Input: part model. Units: mm. Frame: model coordinates. Coordinates: 2 decimals unless noted, no trailing zeros. Write each loop counter-clockwise with the first axis right and the second up, starting at its lowest first coordinate (ties: lowest second). Pieces come first, ordered by that corner, then holes.
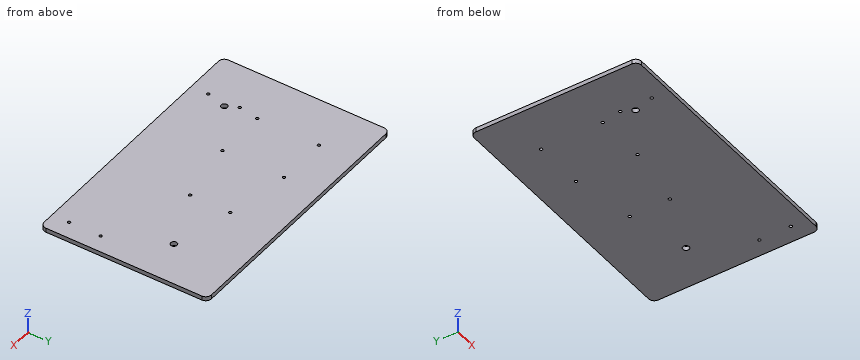
from build123d import *

# Parameters (mm, degrees)
SKETCH_1_R           = 5
SKETCH_1_R_2         = 11
BOSS_EXTRUDE_1_DEPTH = 15


with BuildPart() as part:
    # Sketch 1 → Boss-Extrude 1 (new body)
    with BuildSketch(Plane.XY):
        with BuildLine():
            Line((-465, -273), (-465, 273))
            ThreePointArc((-465, 273), (-459.142135624, 287.142135624), (-445, 293))
            Line((-445, 293), (445, 293))
            ThreePointArc((445, 293), (459.142135624, 287.142135624), (465, 273))
            Line((465, 273), (465, -273))
            ThreePointArc((465, -273), (459.142135624, -287.142135624), (445, -293))
            Line((445, -293), (-445, -293))
            ThreePointArc((-445, -293), (-459.142135624, -287.142135624), (-465, -273))
        make_face()
        with Locations((-115, 163)):
            Circle(SKETCH_1_R, mode=Mode.SUBTRACT)
        with Locations((-293, 163)):
            Circle(SKETCH_1_R, mode=Mode.SUBTRACT)
        with Locations(Location((-293, -53, 0), (0, 0, 180))):
            Circle(SKETCH_1_R, mode=Mode.SUBTRACT)
        with Locations((105, -15)):
            Circle(SKETCH_1_R, mode=Mode.SUBTRACT)
        with Locations(Location((-115, -53, 0), (0, 0, 180))):
            Circle(SKETCH_1_R, mode=Mode.SUBTRACT)
        with Locations(Location((105, 125, 0), (0, 0, 180))):
            Circle(SKETCH_1_R, mode=Mode.SUBTRACT)
        with Locations((-305, -123)):
            Circle(SKETCH_1_R, mode=Mode.SUBTRACT)
        with Locations(Location((-305, -233, 0), (0, 0, 180))):
            Circle(SKETCH_1_R, mode=Mode.SUBTRACT)
        with Locations((405, -233)):
            Circle(SKETCH_1_R, mode=Mode.SUBTRACT)
        with Locations(Location((405, -123, 0), (0, 0, 180))):
            Circle(SKETCH_1_R, mode=Mode.SUBTRACT)
        with Locations((315, 72.5)):
            Circle(SKETCH_1_R_2, mode=Mode.SUBTRACT)
        with Locations((-285, -163)):
            Circle(SKETCH_1_R_2, mode=Mode.SUBTRACT)
    extrude(amount=BOSS_EXTRUDE_1_DEPTH)


solid = part.part
Item 1: Section query A-A, the plane x = 315. Return loops of the section in (y, z), then the cut area to 3 significant figures.
Item 2: Material intervals for line 1 (X direction, y = -53, z = 5.25); line 2 (Y direction, x = -305, z = 10.5); line 3 (Y direction, x = -290.5, z = 10.5), sorted ascending.
Item 3: Section query B-B, the plane y = 72.5. Return loops of the section in (x, z), then the cut area to 3 significant figures.
The answers:
1. outline: (-293, 0) - (61.5, 0) - (61.5, 15) - (-293, 15) - close; (83.5, 0) - (293, 0) - (293, 15) - (83.5, 15) - close
1. area: 8,460 mm2
2. line 1: x = -465 to -298, -288 to -120, -110 to 465
2. line 2: y = -293 to -238, -228 to -128, -118 to 293
2. line 3: y = -293 to -172.53, -153.47 to -57.33, -48.67 to 158.67, 167.33 to 293
3. outline: (-465, 0) - (304, 0) - (304, 15) - (-465, 15) - close; (326, 0) - (465, 0) - (465, 15) - (326, 15) - close
3. area: 13,600 mm2
